Geometry: final body of the model. Coordinates: model frame, mm. Give positions to 0.01 mm unless a question says otherwise; leave off trailing zeros. Loops run counter-clockwise (first coordinate to the right, second up) from the corner with the lowest first, then second, coordinate; pieces in that order, holes last.
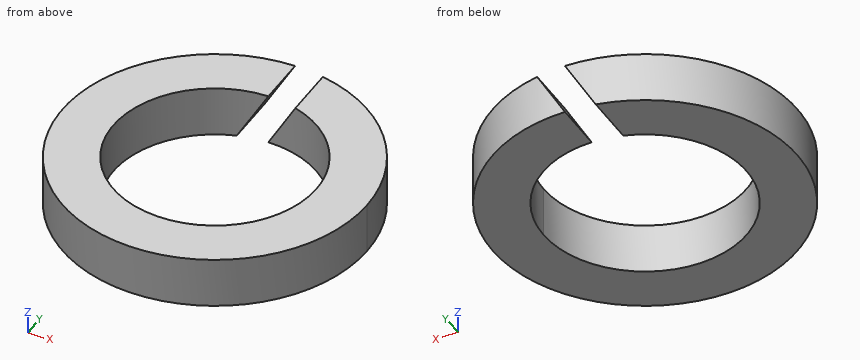
from build123d import *

# Parameters (mm, degrees)
SKETCH1_R          = 3.3
SKETCH1_R_2        = 2.2
BASE_EXTRUDE_DEPTH = 1.1
CUT_EXTRUDE1_DEPTH = 5.794788838


with BuildPart() as part:
    # Sketch1 → Base-Extrude (new body)
    with BuildSketch(Plane.XY):
        Circle(SKETCH1_R)
        Circle(SKETCH1_R_2, mode=Mode.SUBTRACT)
    extrude(amount=-BASE_EXTRUDE_DEPTH)

    # Sketch2 → Cut-Extrude1 (cut, through all)
    with BuildSketch(Plane(origin=(0, 0, 0), x_dir=(1, 0, 0), z_dir=(0, 1, 0))):
        Polygon((0, 1.1), (0.635085296, 0), (0, 0), (-0.635085296, 1.1), align=None)
    extrude(amount=CUT_EXTRUDE1_DEPTH, mode=Mode.SUBTRACT)


solid = part.part
Item 1: Section query D-D on x = 2.75. Return loops of the section in (y, z).
Values follow:
outline: (-1.82, -1.1) - (1.82, -1.1) - (1.82, 0) - (-1.82, 0) - close
Item 2: Ray query, probe 1 along X at (y, z) = (0, -0.85); probe 2 along X at (y, z) = (-2, -0.75); probe 3 along Y at (x, z) = (0, -0.35). Return the intervals inside material, ascending.
Values follow:
probe 1: x = -3.3 to -2.2, 2.2 to 3.3
probe 2: x = -2.62 to -0.92, 0.92 to 2.62
probe 3: y = -3.3 to -2.2
Item 3: Pin query (flat end, axial travel): pin 1 (3 mm diameter, centred on x = 1.5, y = 1.5, fed in from -Z). Return the tip coordinate at first contact, or that it passes through.
Values follow:
pin 1: stops at z = -1.1
Item 4: Section query A-A on y = 0.5. Return loops of the section in (x, z), plus the area to 3 significant figures.
Values follow:
outline: (-3.26, -1.1) - (-2.14, -1.1) - (-2.14, 0) - (-3.26, 0) - close; (2.14, -1.1) - (3.26, -1.1) - (3.26, 0) - (2.14, 0) - close
area: 2.46 mm2
Item 5: Section query C-C on z = -0.25. Return loops of the section in (x, y), plus the area to 3 significant figures.
Values follow:
outline: (-0.14, 2.2) - (-0.14, 3.3) arc R3.3 ccw (long way) to (0.49, 3.26) - (0.49, 2.14) arc R2.2 cw (long way) to start
area: 18.3 mm2
Item 6: Section query B-B on x = -1.5. Return loops of the section in (y, z), plus the area to 3 significant figures.
Values follow:
outline: (-2.94, -1.1) - (-1.61, -1.1) - (-1.61, 0) - (-2.94, 0) - close; (1.61, -1.1) - (2.94, -1.1) - (2.94, 0) - (1.61, 0) - close
area: 2.93 mm2
